```python
from build123d import *

# Parameters (mm, degrees)
SKETCH_2_R   = 12.5
SKETCH_2_R_2 = 10


with BuildPart() as part:
    # 扫描1: sweep along a path in 草图1
    with BuildLine(Plane.XY) as sweep_1_path:
        Line((0, 0), (0, 14))
        ThreePointArc((0, 14), (3.807611845, 23.192388155), (13, 27))
        Line((13, 27), (27, 27))
    # 草图2 → 扫描1 (sweep)
    with BuildSketch(Plane(origin=(0, 0, 0), x_dir=(1, 0, 0), z_dir=(0, 1, 0))):
        Circle(SKETCH_2_R)
        Circle(SKETCH_2_R_2, mode=Mode.SUBTRACT)
    sweep(path=sweep_1_path.line)


solid = part.part
```
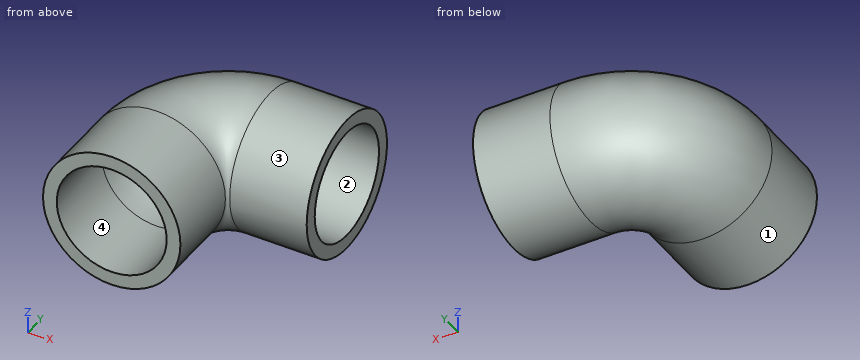
Design review of the part built by this model. Coordinates are the model's own, in mm. Face numbers are marked on the shaded views. A direction names the side the tool comes from. Round coordinates to 2 decimals unless told otherwise and drop trailing zeros. Order: outer loops, then holes, each group sorted by start corner. A loop starts at its lowest first (then second) coordinate and runs counter-clockwise, first axis right, second up. Notation, with made-up numbers: M -29.5,45 L -13.5,45 A25 ccw -13.5,60 Z; hole C -12,53 d8. An arc over 180 degrees is marked long. Put each result on its own line as item: value.
Q1. Consider section A-A (z = 0). State the section outline as (x, y) points, and give its area (3 significant figures).
Reported:
outline: M -12.5,0 L -10,0 L -10,14 A23 cw 13,37 L 27,37 L 27,39.5 L 13,39.5 A25.5 ccw -12.5,14 Z; M 10,0 L 12.5,0 L 12.5,14 A0.5 cw 13,14.5 L 27,14.5 L 27,17 L 13,17 A3 ccw 10,14 Z
area: 242 mm²
Q2. Draft analysis for pull direction Z (two halves, no side actions). For the marked faces 3 and 4, state which applies: released by +Z, released by -Z, zero draft, split by the parting line, or undercut.
Reported:
face 3: split by the parting line
face 4: undercut
Q3. To check wall thickness, follow line 1 (Z direction, x = 17.5, y = 27); line 2 (Y direction, x = 21.75, z = 0); line 3 (Z direction, x = 3.5, y = 27). State the ranges of each line that lie inside material, in increasing order.
Reported:
line 1: -12.5 to -10, 10 to 12.5
line 2: 14.5 to 17, 37 to 39.5
line 3: -12.11 to -9.51, 9.51 to 12.11
Q4. Machinability: for the marked faces 1 and 2, which of the approach directions +Z, -Z, +X, -X, +Y, -Y give a long, thin tool a straight path to every point of the face, cutting with its end or side? Answer none if there is none.
Reported:
face 1: -Y
face 2: +X
Q5. Insertion check: pin 1 Ø5 at (y, z) = (5, 4) entering from +X; pin 2 Ø4 at (x, y) = (13.5, 22) entering from -Z; pin 3 Ø8 at (x, y) = (4.5, 30.5) entering from -Z. Each pin has a flat end and moves straight along its axis. Give the tip position at first contact, or say it passes through.
Reported:
pin 1: x = 12.41
pin 2: z = -12.13
pin 3: z = -12.4
Q6. Consider section B-B (x = 17). State the section outline as (y, z) points.
Reported:
outline: C 27,0 d25; hole C 27,0 d20
Q7. Consider section C-C (y = 6). State the section outline as (x, z) points.
Reported:
outline: C 0,0 d25; hole C 0,0 d20
